from build123d import *

# Parameters (mm, degrees)
SKETCH1_W             = 80
SKETCH1_H             = 320
BOSS_EXTRUDE1_DEPTH   = 12.5
M8_TAPPED_HOLE1_D     = 6.8
M8_TAPPED_HOLE1_DEPTH = 19.75
M8_TAPPED_HOLE1_TIP   = 2.042926105
CHAMFER1_SIZE         = 2
M4_TAPPED_HOLE1_D     = 3.3
M4_TAPPED_HOLE1_DEPTH = 10.1
M4_TAPPED_HOLE1_TIP   = 0.991420021
M8_TAPPED_HOLE2_D     = 6.8
M8_TAPPED_HOLE2_DEPTH = 19.75
M8_TAPPED_HOLE2_TIP   = 2.042926105
CUT_EXTRUDE2_DEPTH    = 15


with BuildPart() as part:
    # Sketch1 → Boss-Extrude1 (new, symmetric)
    with BuildSketch(Plane(origin=(0, 0, 0), x_dir=(1, 0, 0), z_dir=(0, 1, 0))):
        with Locations((40, 160)):
            Rectangle(SKETCH1_W, SKETCH1_H)
    extrude(amount=BOSS_EXTRUDE1_DEPTH, both=True)

    # M8 Tapped Hole1
    with Locations(Plane.XY):
        with Locations((15, 0), (65, 0)):
            Hole(M8_TAPPED_HOLE1_D / 2, depth=M8_TAPPED_HOLE1_DEPTH)
            with Locations((0, 0, -(M8_TAPPED_HOLE1_DEPTH + M8_TAPPED_HOLE1_TIP / 2))):  # 118° drill point
                Cone(0, M8_TAPPED_HOLE1_D / 2, M8_TAPPED_HOLE1_TIP, mode=Mode.SUBTRACT)

    # Chamfer1
    chamfer1_edges = [part.edges().sort_by_distance(p)[0] for p in [
        (0, 0, -320),
        (80, 0, -320),
    ]]
    chamfer(chamfer1_edges, length=CHAMFER1_SIZE)

    # M4 Tapped Hole1
    with Locations(Plane(origin=(0, 12.5, 0), x_dir=(1, 0, 0), z_dir=(0, 1, 0))):
        with Locations((30, 305), (30, 291), (50, 291), (50, 305)):
            Hole(M4_TAPPED_HOLE1_D / 2, depth=M4_TAPPED_HOLE1_DEPTH)
            with Locations((0, 0, -(M4_TAPPED_HOLE1_DEPTH + M4_TAPPED_HOLE1_TIP / 2))):  # 118° drill point
                Cone(0, M4_TAPPED_HOLE1_D / 2, M4_TAPPED_HOLE1_TIP, mode=Mode.SUBTRACT)

    # M8 Tapped Hole2
    with Locations(Plane(origin=(0, 0, -320), x_dir=(-1, 0, 0), z_dir=(0, 0, -1))):
        with Locations((-15, 0), (-65, 0)):
            Hole(M8_TAPPED_HOLE2_D / 2, depth=M8_TAPPED_HOLE2_DEPTH)
            with Locations((0, 0, -(M8_TAPPED_HOLE2_DEPTH + M8_TAPPED_HOLE2_TIP / 2))):  # 118° drill point
                Cone(0, M8_TAPPED_HOLE2_D / 2, M8_TAPPED_HOLE2_TIP, mode=Mode.SUBTRACT)

    # Sketch11 → Cut-Extrude2 (cut)
    with BuildSketch(Plane.XZ.offset(12.5)):
        with BuildLine():
            Line((50.25, -160), (50.25, -320))
            ThreePointArc((50.25, -320), (40, -330.25), (29.75, -320))
            Line((29.75, -320), (29.75, -160))
            ThreePointArc((29.75, -160), (40, -149.75), (50.25, -160))
        make_face()
    extrude(amount=-CUT_EXTRUDE2_DEPTH, mode=Mode.SUBTRACT)


solid = part.part
Work out the finished part from the listing and answer in its coordinate system (mm). A direction names the side the tool comes from. Coordinates: 2 decimals unless noted, no trailing zeros. Order: outer loops, then holes, each group sorted by start corner. A loop starts at its lowest first (then second) coordinate and runs counter-clockwise, first axis right, second up. Notation, with made-up numbers: (11.5, 66.25) - (32.5, 66.25) arc R26 cw to (32.5, 91.25) - close; hole circle Ø8 at (72, 61.25). An arc over 180 degrees is marked (long way). Put each result on its own line as item: value. Start each with the question number.
1) For faces 1 (the flat face through (29.75, -5, -241)), 2 (the cylindrical face through (61.86, -1.3, -10.01)), 3 (the flat face through (0, 0, -157)), 4 (the flat face through (39, 0, 0)), 5 (the cylindrical face through (68.243, 1.021, -309.987)), determine the directions among +Z, -Z, +X, -X, +Y, -Y from which every point of the face is accessible in a straight line to the end or side of a thin tool.
2) For a pull along X with two mould halves and no side action, classify faces 6 (the flat face through (80, 0, -157)), 7 (the flat face through (39, -12.5, -127)), 8 (the cylindrical face through (17.698, -2.069, -10.013)) as released by +X, released by -X, zero draft, split by the parting line, or undercut.
3) Find section A-A (z = -240). Give the vertices of the cut face in (x, y), plus the area to 3 significant figures.
4) Find the intervals of material crossed by line 1 (X direction, y = 0, z = -7.5); line 2 (Z direction, x = 50, y = 6.5); line 3 (X direction, y = 9, z = -305), in increasing order. Write a range as from..to.
5) Flat-ended cylindrical pins translate along their axes: pin 1 (2.5 mm diameter, centred on x = 50, z = -305, fed in from +Y); pin 2 (4 mm diameter, centred on x = 15, y = 0, fed in from -Z); pin 3 (4 mm diameter, centred on x = 65, y = 0, fed in from +Z). Find the tip coordinate at first contact, or state that the pin passes through.
6) Find section B-B (y = -6.25). Give the vertices of the cut face in (x, z), plus the area to 3 significant figures.
Results list:
1. face 1: -Z, -Y
1. face 2: +Z
1. face 3: +Z, -Z, -X, +Y, -Y
1. face 4: +Z, +X, -X, +Y, -Y
1. face 5: -Z
2. face 6: released by +X
2. face 7: zero draft
2. face 8: undercut
3. outline: (0, -12.5) - (29.75, -12.5) - (29.75, 2.5) - (50.25, 2.5) - (50.25, -12.5) - (80, -12.5) - (80, 12.5) - (0, 12.5) - close
3. area: 1,690 mm^2
4. line 1: x = 0..11.6, 18.4..61.6, 68.4..80
4. line 2: z = -320..-306.65, -303.35..-292.65, -289.35..0
4. line 3: x = 0..28.35, 31.65..48.35, 51.65..80
5. pin 1: stops at y = 2.16
5. pin 2: stops at z = -299.41
5. pin 3: stops at z = -20.59
6. outline: (0, -318) - (2, -320) - (29.75, -320) - (29.75, -160) arc R10.25 cw to (50.25, -160) - (50.25, -320) - (78, -320) - (80, -318) - (80, 0) - (0, 0) - close
6. area: 22,200 mm^2
